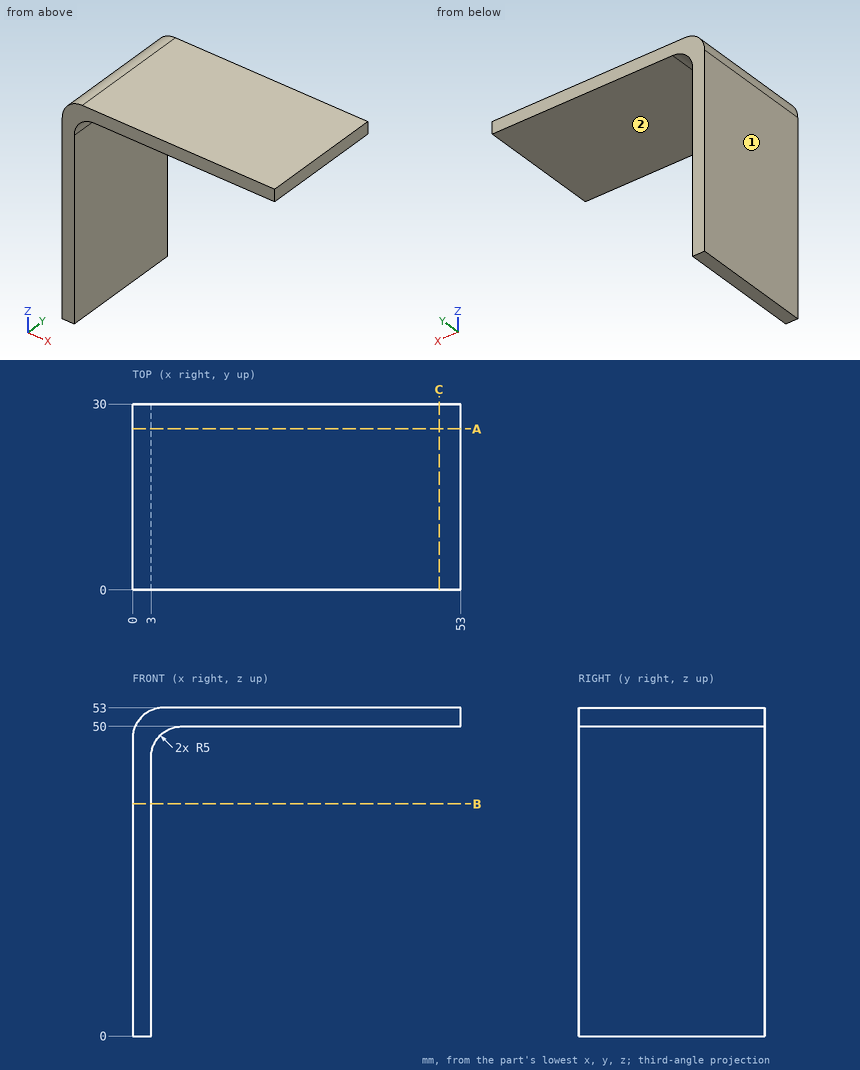
For this review, use the dimensioned drawing (mm, ordinates from the lowest corner) and the shaded views. A direction names the side the tool comes from. Round coordinates to 2 decimals unless told otherwise and drop trailing zeros. Write each loop counter-clockwise with the first axis right and the second up, starting at its lowest first coordinate (ties: lowest second). Pieces come first, ordered by that corner, then holes. Notation, with made-up numbers: (49.25, 22) - (103.25, 22) arc R25 cw to (103.25, 41) - close; hole circle Ø10 at (-38, 11.25). An arc over 180 degrees is marked (long way). One line per item, written item: value. Start each with the question number.
1. Clearance check with flat-ended pins moving along their axes: P1, Ø10, axis at y = 22, z = 8.5, coming from the +X side; P2, Ø9, axis at x = 21, y = 10, coming from the -Z side. State where each tip first meets the part, or that it passes through.
2. To check wall thickness, follow L1, parallel to X at y = 2.75, z = 39; L2, parallel to Z at x = 42, y = 18.5; L3, parallel to Z at x = 4, y = 8. State the ranges of each line that lie inside material, in increasing order. Write a range as from..to.
3. Consider section A-A on y = 26. Write out the cut boundary in (x, z), and give its area (3 significant figures).
4. Machinability: for the marked faces 1 and 2, which of the approach directions +Z, -Z, +X, -X, +Y, -Y give a long, thin tool a straight path to every point of the face, cutting with its end or side? Answer none if there is none.
5. Consider section C-C on x = 49.5. Write out the cut boundary in (y, z), and give its area (3 significant figures).
6. Consider section B-B on z = 37.5. Write out the cut boundary in (x, y), and give its area (3 significant figures).
Checks:
1. P1: stops at x = 3
1. P2: stops at z = 50
2. L1: x = 0..3
2. L2: z = 50..53
2. L3: z = 48..52.9
3. outline: (0, 0) - (3, 0) - (3, 45) arc R5 cw to (8, 50) - (53, 50) - (53, 53) - (5, 53) arc R5 ccw to (0, 48) - close
3. area: 309 mm^2
4. face 1: +Z, -Z, -X, +Y, -Y
4. face 2: -Z, +X, +Y, -Y
5. outline: (0, 50) - (30, 50) - (30, 53) - (0, 53) - close
5. area: 90.0 mm^2
6. outline: (0, 0) - (3, 0) - (3, 30) - (0, 30) - close
6. area: 90.0 mm^2
